```python
from build123d import *

# Parameters (mm, degrees)
FLANGE_DISC_PROFILE_R          = 150
FLANGE_DISC_300_DEPTH          = 30
RAISED_FACE_PROFILE_R          = 97.5
RAISED_FACE_195_DEPTH          = 8
HUB_SPIGOT_PROFILE_R           = 40.15
HUB_SPIGOT_80_3_DEPTH          = 2
THROUGH_HOLES_PROFILE_R        = 6
THROUGH_HOLES_PROFILE_R_2      = 11.75
THROUGH_HOLES_PCD254_DEPTH     = 40
COUNTERBORE_PROFILE_R          = 17.5
COUNTERBORES_4X_35_DEPTH       = 16
COUNTERBORED_HOLES_PROFILE_R   = 11.5
COUNTERBORED_HOLES_4X_23_DEPTH = 30
CENTRAL_BORE_PROFILE_R         = 35
CENTRAL_BORE_70_DEPTH          = 50


with BuildPart() as part:
    # Flange Disc Profile → Flange Disc Ø300 (new body)
    with BuildSketch(Plane.XY):
        Circle(FLANGE_DISC_PROFILE_R)
    extrude(amount=FLANGE_DISC_300_DEPTH)

    # Raised Face Profile → Raised Face Ø195 (add)
    with BuildSketch(Plane.XY.offset(30)):
        Circle(RAISED_FACE_PROFILE_R)
    extrude(amount=RAISED_FACE_195_DEPTH)

    # Hub Spigot Profile → Hub Spigot Ø80.3 (add)
    with BuildSketch(Plane.XY.offset(38)):
        Circle(HUB_SPIGOT_PROFILE_R)
    extrude(amount=HUB_SPIGOT_80_3_DEPTH)

    # Through Holes Profile → Through Holes PCD254 (cut)
    with BuildSketch(Plane.XY.offset(40)):
        with Locations((-60, 60)):
            Circle(THROUGH_HOLES_PROFILE_R)
        with Locations((89.802561211, 89.802561211)):
            Circle(THROUGH_HOLES_PROFILE_R_2)
        with Locations((89.802561211, -89.802561211)):
            Circle(THROUGH_HOLES_PROFILE_R_2)
        with Locations((-89.802561211, -89.802561211)):
            Circle(THROUGH_HOLES_PROFILE_R_2)
        with Locations((-89.802561211, 89.802561211)):
            Circle(THROUGH_HOLES_PROFILE_R_2)
    extrude(amount=-THROUGH_HOLES_PCD254_DEPTH, mode=Mode.SUBTRACT)

    # Counterbore Profile → Counterbores 4xØ35 (cut)
    with BuildSketch(Plane.XY.offset(38)):
        with Locations((-28.338059011, 69.440293861)):
            Circle(COUNTERBORE_PROFILE_R)
        with Locations((69.440293861, 28.338059011)):
            Circle(COUNTERBORE_PROFILE_R)
        with Locations((28.338059011, -69.440293861)):
            Circle(COUNTERBORE_PROFILE_R)
        with Locations((-69.440293861, -28.338059011)):
            Circle(COUNTERBORE_PROFILE_R)
    extrude(amount=-COUNTERBORES_4X_35_DEPTH, mode=Mode.SUBTRACT)

    # Counterbored Holes Profile → Counterbored Holes 4xØ23 (cut)
    with BuildSketch(Plane.XY.offset(22)):
        with Locations((-28.338059011, 69.440293861)):
            Circle(COUNTERBORED_HOLES_PROFILE_R)
        with Locations((69.440293861, 28.338059011)):
            Circle(COUNTERBORED_HOLES_PROFILE_R)
        with Locations((28.338059011, -69.440293861)):
            Circle(COUNTERBORED_HOLES_PROFILE_R)
        with Locations((-69.440293861, -28.338059011)):
            Circle(COUNTERBORED_HOLES_PROFILE_R)
    extrude(amount=-COUNTERBORED_HOLES_4X_23_DEPTH, mode=Mode.SUBTRACT)

    # Central Bore Profile → Central Bore Ø70 (cut)
    with BuildSketch(Plane.XY.offset(40)):
        Circle(CENTRAL_BORE_PROFILE_R)
    extrude(amount=-CENTRAL_BORE_70_DEPTH, mode=Mode.SUBTRACT)


solid = part.part
```
For this review, take the finished solid that the model builds, in its own axes (mm). A direction names the side the tool comes from. Coordinates: 2 decimals unless noted, no trailing zeros. Loops run counter-clockwise (first coordinate to the right, second up) from the corner with the lowest first, then second, coordinate; pieces in that order, holes last.
1. Add section A-A, the plane y = 0. Give the boundary of the cut face in (x, z), then the cut area to 3 significant figures.
2. For line 1 (X direction, y = 62, z = 31); line 2 (Y direction, x = -92, z = 24); line 3 (X direction, y = -80, z = 4.5), list the stretches that pass through material, from the lowest coordinate up.
3. Add section C-C, the plane z = 17. Count the separate pieces of the cut face and the enclosed holes in it, then the cut area to 3 significant figures.
4. Mouldability with a two-part tool opening along X and no side actions: class faces 1 (the cylindrical face through (-84.381, -100.227, 15.21)), 2 (the cylindrical face through (80.41, 31.79, 11.15)), 3 (the cylindrical face through (-77.37, -59.33, 33.94)), 4 (the flat face through (-1, -42, 38)) as +X half, -X half, draft (parallel to the pull), parting line (faces both ways), or undercut.
5. For faces 5 (the cylindrical face through (-30.831, 58.214, 11.154)), 6 (the cylindrical face through (-32.132, 52.356, 30.112)), list the 3-axis set-ups (+Z, -Z, +X, -X, +Y, -Y) from which the entire face can be reached by the end or side of a thin tool; tool diameter is ignored.
6. Insertion check: P1, Ø3, axis at x = 53, z = 18, coming from the -Y side; P2, Ø10, axis at x = -47.5, z = 20.5, coming from the -Y side; P3, Ø2, axis at x = 77, y = -22, coming from the +Z side; P4, Ø1, axis at x = 35, y = 44.5, coming from the -Z side. Each pin has a flat end and moves straight along its axis. Give the tip position at first contact, or say it passes through.
7. Add section D-D, the plane z = 34. Give the boundary of the cut face in (x, y).
Result:
1. outline: (-150, 0) - (-35, 0) - (-35, 40) - (-40.15, 40) - (-40.15, 38) - (-97.5, 38) - (-97.5, 30) - (-150, 30) - close; (35, 0) - (150, 0) - (150, 30) - (97.5, 30) - (97.5, 38) - (40.15, 38) - (40.15, 40) - (35, 40) - close
1. area: 7,920 mm2
2. line 1: x = -75.25 to -65.66, -54.34 to -44.18, -12.5 to 75.25
2. line 2: y = -118.47 to -101.35, -78.26 to 78.26, 101.35 to 118.47
2. line 3: x = -126.89 to -96.28, -83.32 to 23.78, 32.89 to 83.32, 96.28 to 126.89
3. separate pieces: 1
3. enclosed holes: 10
3. area: 63,300 mm2
4. face 1: undercut
4. face 2: undercut
4. face 3: parting line
4. face 4: draft
5. face 5: +Z, -Z
5. face 6: +Z
6. P1: stops at y = -140.88
6. P2: stops at y = -143.85
6. P3: stops at z = 38
6. P4: stops at z = 0
7. outline: circle Ø195 at (0, 0); hole circle Ø35 at (-69.44, -28.34); hole circle Ø12 at (-60, 60); hole circle Ø35 at (-28.34, 69.44); hole circle Ø70 at (0, 0); hole circle Ø35 at (28.34, -69.44); hole circle Ø35 at (69.44, 28.34)
